```python
from build123d import *

# Parameters (mm, degrees)
SKETCH_1_R      = 1.25
EXTRUDE_1_DEPTH = 1.2


with BuildPart() as part:
    # 草图1 → 凸台-拉伸1 (new, symmetric)
    with BuildSketch(Plane.XY):
        Polygon((3.175426481, 0), (1.58771324, 2.75), (-1.58771324, 2.75), (-3.175426481, 0), (-1.58771324, -2.75), (1.58771324, -2.75), align=None)
        Circle(SKETCH_1_R, mode=Mode.SUBTRACT)
    extrude(amount=EXTRUDE_1_DEPTH, both=True)


solid = part.part
```
CAD build for the part. Positions are in the model's coordinates, mm. Round coordinates to 2 decimals unless told otherwise and drop trailing zeros. Loops run counter-clockwise (first coordinate to the right, second up) from the corner with the lowest first, then second, coordinate; pieces in that order, holes last. Notation, with made-up numbers: (-19.5, 65.5) - (-14.5, 65.5) arc R32 ccw to (-14.5, 93.5) - close; hole circle Ø6 at (60, -37). An arc over 180 degrees is marked (long way). Return JSON: item names as keys, results as strings. Group by question number.
Q1. Band-saw the part on B-B on z = 1. Give the cut face in (x, y).
Q2. Flat gauge pin, fed straight in: pin 1 Ø1 at (y, z) = (-1.5, 0.5) entering from -X. Where does the tip first touch, or does it go through?
Q3. Two-plate mould, pull along X, no slides. Class faces 1 (the face through (0, -2.75, 0)), 2 (the face through (-2.39, -1.36, 0.02)), 3 (the face through (-0.27, -1.22, -0.02)): +X half, -X half, draft (parallel to the pull), parting line (faces both ways), or undercut.
Q4. Band-saw the part on C-C on y = 0.75. Give the cut face in (x, z), plus the area to 3 significant figures.
Q5. Band-saw the part on A-A on x = 0. Give the cut face in (y, z), plus the area to 3 significant figures.
Q6. Drill centre lines: line 1 along Y through (x, z) = (0, 0.15); line 2 along X through (y, z) = (0.2, 0.9); line 3 along Y through (x, z) = (-0.75, 0.35). Where is each one in solid material? Low to high. Write a range as [from, to].
Q7. Band-saw the part on D-D on x = 1.75. Give the cut face in (y, z), plus the area to 3 significant figures.
Solutions:
{
 "1": {"outline": "(-3.18, 0) - (-1.59, -2.75) - (1.59, -2.75) - (3.18, 0) - (1.59, 2.75) - (-1.59, 2.75) - close; hole circle Ø2.5 at (0, 0)"},
 "2": {"pin 1": "stops at x = -2.6"},
 "3": {"face 1": "draft", "face 2": "-X half", "face 3": "undercut"},
 "4": {"outline": "(-2.74, -1.2) - (-1, -1.2) - (-1, 1.2) - (-2.74, 1.2) - close; (1, -1.2) - (2.74, -1.2) - (2.74, 1.2) - (1, 1.2) - close", "area": "8.36 mm^2"},
 "5": {"outline": "(-2.75, -1.2) - (-1.25, -1.2) - (-1.25, 1.2) - (-2.75, 1.2) - close; (1.25, -1.2) - (2.75, -1.2) - (2.75, 1.2) - (1.25, 1.2) - close", "area": "7.20 mm^2"},
 "6": {"line 1": "y = [-2.75, -1.25], [1.25, 2.75]", "line 2": "x = [-3.06, -1.23], [1.23, 3.06]", "line 3": "y = [-2.75, -1], [1, 2.75]"},
 "7": {"outline": "(-2.47, -1.2) - (2.47, -1.2) - (2.47, 1.2) - (-2.47, 1.2) - close", "area": "11.9 mm^2"}
}
